from build123d import *

# Parameters (mm, degrees)
EXTRUDE_1_DEPTH     = 10
SKETCH_10_R         = 2.5
SKETCH_10_R_2       = 2.1
CUT_EXTRUDE_1_DEPTH = 10
SKETCH_11_R         = 5.5
CUT_EXTRUDE_2_DEPTH = 5


with BuildPart() as part:
    # 草图1 → 凸台-拉伸1 (new body)
    with BuildSketch(Plane.XY):
        Polygon((-99.58041958, -70.769230769), (-39.58041958, -70.769230769), (-39.58041958, -100.769230769), (40.41958042, -100.769230769), (40.41958042, 299.230769231), (-99.58041958, 299.230769231), align=None)
    extrude(amount=EXTRUDE_1_DEPTH)

    # 草图10 → 切除-拉伸1 (cut)
    with BuildSketch(Plane.XY.offset(10)):
        with Locations((-79.008794304, 258.253022412)):
            Circle(SKETCH_10_R)
        with Locations((20.991205696, 258.253022412)):
            Circle(SKETCH_10_R)
        with Locations((-50.330419577, 211.582541175)):
            Circle(SKETCH_10_R_2)
        with Locations((-50.330419577, 189.082541175)):
            Circle(SKETCH_10_R_2)
        with Locations((10.169580423, 211.582541175)):
            Circle(SKETCH_10_R_2)
        with Locations((10.169580423, 189.082541175)):
            Circle(SKETCH_10_R_2)
        with Locations((-42.717061736, -29.519230769)):
            Circle(SKETCH_10_R_2)
        with Locations((-42.717061736, -57.019230769)):
            Circle(SKETCH_10_R_2)
        with Locations((12.707366369, -57.019230769)):
            Circle(SKETCH_10_R_2)
        with Locations((12.707366369, -29.519230769)):
            Circle(SKETCH_10_R_2)
        with Locations((20.991205696, 18.253022412)):
            Circle(SKETCH_10_R)
    extrude(amount=-CUT_EXTRUDE_1_DEPTH, mode=Mode.SUBTRACT)

    # 草图11 → 切除-拉伸2 (cut)
    with BuildSketch(Plane(origin=(-949.724352481, 990.975018952, 10), x_dir=(0, -1, 0), z_dir=(0, 0, 1))):
        with Locations(Location((732.680785462, 870.715566681, 0), (0, 0, 90))):
            Circle(SKETCH_11_R)
        with Locations(Location((732.72199654, 970.71555819, 0), (0, 0, 90))):
            Circle(SKETCH_11_R)
        with Locations(Location((972.72199654, 970.71555819, 0), (0, 0, 90))):
            Circle(SKETCH_11_R)
    extrude(amount=-CUT_EXTRUDE_2_DEPTH, mode=Mode.SUBTRACT)


solid = part.part
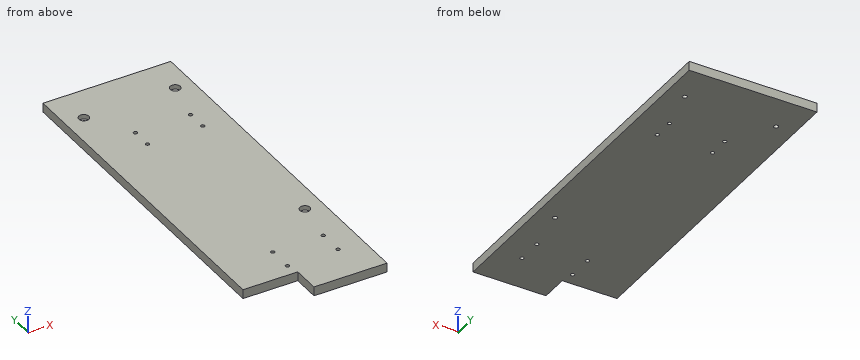
Here's how the part is built. I have some questions about the finished solid (model axes, mm). Give positions to 0.01 mm unless a question says otherwise; leave off trailing zeros. Order: outer loops, then holes, each group sorted by start corner. A loop starts at its lowest first (then second) coordinate and runs counter-clockwise, first axis right, second up. Notation, with made-up numbers: (-35.5, 47) -> (-5.5, 47) arc R13 ccw to (-5.5, 54) -> close; hole circle Ø6 at (64, -25). An arc over 180 degrees is marked (long way). Use a Markdown table: item, result. Add a question column.
Item 1: Imagine slicing it at B-B on x = -89.5. Please give me the cut outline in (y, z), plus the area to 3 significant figures.
Item 2: I need wall thicknesses on line 1 (Y direction, x = -42.5, z = 6.25); line 2 (Y direction, x = 9, z = 9); line 3 (Y direction, x = -90, z = 3). Which ranges of each line are inside material? Lowest first, please.
Item 3: Imagine slicing it at A-A on z = 3.25. Give the number of separate pieces and of enclosed holes in the cut face, plus the area to 3 significant figures.
Item 4: Will these pins go through, and if not, where does the flat tip stop? pin 1 (2 mm diameter, centred on x = -76.5, z = 8, fed in from -Y); pin 2 (5.5 mm diameter, centred on x = 22.5, y = 17, fed in from +Z); pin 3 (4 mm diameter, centred on x = 10.17, y = 189.08, fed in from +Z).
Data:
| question | item | result |
|---|---|---|
| 1 | outline | (-70.77, 0) -> (299.23, 0) -> (299.23, 10) -> (-70.77, 10) -> close |
| 1 | area | 3,700 mm² |
| 2 | line 1 | y = -70.77 to -59.11, -54.93 to -31.61, -27.43 to 299.23 |
| 2 | line 2 | y = -100.77 to 187.34, 190.83 to 209.84, 213.33 to 299.23 |
| 2 | line 3 | y = -70.77 to 299.23 |
| 3 | separate pieces | 1 |
| 3 | enclosed holes | 11 |
| 3 | area | 54,000 mm² |
| 4 | pin 1 | stops at y = -70.77 |
| 4 | pin 2 | stops at z = 5 |
| 4 | pin 3 | passes through |
